```python
from build123d import *

# Parameters (mm, degrees)
SKETCH1_R             = 6
BOSS_EXTRUDE1_DEPTH   = 44
SKETCH2_W             = 70
SKETCH2_H             = 68
CUT_EXTRUDE1_DEPTH    = 142.194900758
CUT_EXTRUDE2_DEPTH    = 142.194900758
M4_TAPPED_HOLE1_D     = 3.3
M4_TAPPED_HOLE1_DEPTH = 10.1
M4_TAPPED_HOLE1_TIP   = 0.991420021
SKETCH7_W             = 45
SKETCH7_H             = 64
CUT_EXTRUDE4_DEPTH    = 142.194900874
SKETCH8_W             = 48
SKETCH8_H             = 20
CUT_EXTRUDE5_DEPTH    = 142.194900874
CHAMFER1_SIZE         = 5
CHAMFER2_SIZE         = 2
CHAMFER3_SIZE         = 1
FILLET1_R             = 5


with BuildPart() as part:
    # Sketch1 → Boss-Extrude1 (new, symmetric)
    with BuildSketch(Plane.XY):
        Polygon((0, 0), (0, 60), (120, 60), (120, 40), (15, 40), (15, 0), align=None)
        with Locations((110, 50)):
            Circle(SKETCH1_R, mode=Mode.SUBTRACT)
    extrude(amount=BOSS_EXTRUDE1_DEPTH, both=True)

    # Sketch2 → Cut-Extrude1 (cut, through all)
    with BuildSketch(Plane(origin=(0, 60, 0), x_dir=(1, 0, 0), z_dir=(0, 1, 0))):
        with Locations((120, 0)):
            Rectangle(SKETCH2_W, SKETCH2_H)
    extrude(amount=-CUT_EXTRUDE1_DEPTH, mode=Mode.SUBTRACT)

    # Sketch3 → Cut-Extrude2 (cut, through all)
    with BuildSketch(Plane.ZY):
        with BuildLine():
            Line((-33.5, 6), (-33.5, 11))
            ThreePointArc((-33.5, 11), (-30, 14.5), (-26.5, 11))
            Line((-26.5, 11), (-26.5, 6))
            ThreePointArc((-26.5, 6), (-30, 2.5), (-33.5, 6))
        make_face()
        with BuildLine():
            Line((33.5, 6), (33.5, 11))
            ThreePointArc((33.5, 11), (30, 14.5), (26.5, 11))
            Line((26.5, 11), (26.5, 6))
            ThreePointArc((26.5, 6), (30, 2.5), (33.5, 6))
        make_face()
    extrude(amount=-CUT_EXTRUDE2_DEPTH, mode=Mode.SUBTRACT)

    # M4 Tapped Hole1
    with Locations(Plane(origin=(120, 0, 0), x_dir=(0, 0, -1), z_dir=(1, 0, 0))):
        with Locations((-39, 50), (39, 50)):
            Hole(M4_TAPPED_HOLE1_D / 2, depth=M4_TAPPED_HOLE1_DEPTH)
            with Locations((0, 0, -(M4_TAPPED_HOLE1_DEPTH + M4_TAPPED_HOLE1_TIP / 2))):  # 118° drill point
                Cone(0, M4_TAPPED_HOLE1_D / 2, M4_TAPPED_HOLE1_TIP, mode=Mode.SUBTRACT)

    # Sketch7 → Cut-Extrude4 (cut, through all)
    with BuildSketch(Plane(origin=(0, 60, 0), x_dir=(-1, 0, 0), z_dir=(0, 1, 0))):
        with Locations((-42.5, 0)):
            Rectangle(SKETCH7_W, SKETCH7_H)
    extrude(amount=-CUT_EXTRUDE4_DEPTH, mode=Mode.SUBTRACT)

    # Sketch8 → Cut-Extrude5 (cut, through all)
    with BuildSketch(Plane.ZY):
        with Locations((0, 30)):
            Rectangle(SKETCH8_W, SKETCH8_H)
    extrude(amount=-CUT_EXTRUDE5_DEPTH, mode=Mode.SUBTRACT)

    # Chamfer1
    chamfer1_edges = [part.edges().sort_by_distance(p)[0] for p in [
        (0, 60, 0),
    ]]
    chamfer(chamfer1_edges, length=CHAMFER1_SIZE)

    # Chamfer2
    chamfer2_edges = [part.edges().sort_by_distance(p)[0] for p in [
        (7.5, 0, 44),
        (7.5, 0, -44),
    ]]
    chamfer(chamfer2_edges, length=CHAMFER2_SIZE)

    # Chamfer3
    chamfer3_edges = [part.edges().sort_by_distance(p)[0] for p in [
        (120, 60, 39),
        (120, 40, 39),
        (120, 60, -39),
        (120, 40, -39),
    ]]
    chamfer(chamfer3_edges, length=CHAMFER3_SIZE)

    # Fillet1
    fillet1_edges = [part.edges().sort_by_distance(p)[0] for p in [
        (7.5, 40, 24),
        (7.5, 20, 24),
        (7.5, 20, -24),
        (7.5, 40, -24),
        (85, 50, 34),
        (85, 50, -34),
        (65, 50, -32),
        (65, 50, 32),
        (20, 50, 32),
        (20, 50, -32),
    ]]
    fillet(fillet1_edges, radius=FILLET1_R)


solid = part.part
```
Build history of the part. All positions in model axes, mm. A direction names the side the tool comes from. Give positions to 0.01 mm unless a question says otherwise; leave off trailing zeros. Order: outer loops, then holes, each group sorted by start corner. A loop starts at its lowest first (then second) coordinate and runs counter-clockwise, first axis right, second up. Notation, with made-up numbers: M -17.75,3 L 22.25,3 A23 ccw 22.25,34 Z; hole C -2,-33 d9. An arc over 180 degrees is marked long. Write item = value, one per line. Start each with the question number.
(1) Two-plate mould, pull along X, no slides. Class faces 1 (the cylindrical face through (64, 50, 30)), 2 (the flat face through (120, 52, 39)), 3 (the flat face through (72, 40, -1)), 4 (the flat face through (3, 58, 1)): released by +X, released by -X, zero draft, split by the parting line, or undercut.
(2) Slice it at D-D on x = 110. Write the cut outline in (y, z).
(3) Slice it at C-C on y = 29. Write the cut outline in (x, z), plus the area to 3 significant figures.
(4) Slice it at B-B on x = 51.5. Write the cut outline in (y, z), plus the area to 3 significant figures.
(5) Which spindle directions (+Z, -Z, +X, -X, +Y, -Y) get a long thin tool onto all of the face, cutting with end or side? Do faces 5 (the flat face through (65, 50, 0)), 6 (the cylindrical face through (117.9, 48.4, 38.6)), 7 (the flat face through (101, 50, -34)), 8 (the flat face through (7, 8, 33.5)), 9 (the flat face through (8, 0, 1)). Say none if no direction does.
(6) Slice it at A-A on z = 2. Write the cut outline in (x, y).
(7) Probe L1, parallel to X at y = 48, z = 1.5; L2, parallel to Y at x = 110, z = -40.5; L3, parallel to Z at x = 60.5, y = 41. List the from-to ranges inside material, lowest first. Write a range as [from, to].
(8) Pin check, flat tips, straight feed: pin 1 Ø1 at (y, z) = (42, 27) entering from +X; pin 2 Ø10 at (x, z) = (82.5, -29) entering from -Y. Stop position of each tip, or through.
Responses:
q1.face_1 = undercut
q1.face_2 = released by +X
q1.face_3 = zero draft
q1.face_4 = released by -X
q2.outline = M 40,-44 L 44,-44 L 44,-34 L 40,-34 Z; M 40,34 L 44,34 L 44,44 L 40,44 Z; M 56,-44 L 60,-44 L 60,-34 L 56,-34 Z; M 56,34 L 60,34 L 60,44 L 56,44 Z
q3.outline = M 0,-44 L 15,-44 L 15,-24 L 0,-24 Z; M 0,24 L 15,24 L 15,44 L 0,44 Z
q3.area = 600 mm2
q4.outline = M 40,-44 L 60,-44 L 60,-32 L 40,-32 Z; M 40,32 L 60,32 L 60,44 L 40,44 Z
q4.area = 480 mm2
q5.face_5 = +Y, -Y
q5.face_6 = +X
q5.face_7 = +X, +Y, -Y
q5.face_8 = +X, -X
q5.face_9 = +Z, -Z, +X, -X, -Y
q6.outline = M 0,0 L 15,0 L 15,20 L 0,20 Z; M 0,40 L 20,40 L 20,60 L 5,60 L 0,55 Z; M 65,40 L 85,40 L 85,60 L 65,60 Z
q7.L1 = [0, 20], [65, 85]
q7.L2 = [40, 44], [56, 60]
q7.L3 = [-44, -31.97], [31.97, 44]
q8.pin_1 = 85
q8.pin_2 = 40
